from build123d import *

# Parameters (mm, degrees)
SKETCH1_W           = 50
SKETCH1_H           = 12
BOSS_EXTRUDE1_DEPTH = 5
SKETCH2_R           = 2.25
CUT_EXTRUDE1_DEPTH  = 52.662365412
SKETCH3_W           = 2
SKETCH3_H           = 5
CUT_EXTRUDE2_DEPTH  = 52.662365412
CHAMFER1_SIZE       = 1
MOVE_FACE1_BY       = 6.5


with BuildPart() as part:
    # Sketch1 → Boss-Extrude1 (new body)
    with BuildSketch(Plane.XY):
        with Locations((25, 6)):
            Rectangle(SKETCH1_W, SKETCH1_H)
    extrude(amount=BOSS_EXTRUDE1_DEPTH)

    # Sketch2 → Cut-Extrude1 (cut, through all)
    with BuildSketch(Plane.XY.offset(5)):
        with Locations((10, 8.5)):
            Circle(SKETCH2_R)
        with Locations((40, 8.5)):
            Circle(SKETCH2_R)
    extrude(amount=-CUT_EXTRUDE1_DEPTH, mode=Mode.SUBTRACT)

    # Sketch3 → Cut-Extrude2 (cut, through all)
    with BuildSketch(Plane(origin=(50, 0, 0), x_dir=(0, 0, -1), z_dir=(1, 0, 0))):
        with Locations((-4, 2.5)):
            Rectangle(SKETCH3_W, SKETCH3_H)
    extrude(amount=-CUT_EXTRUDE2_DEPTH, mode=Mode.SUBTRACT)

    # Chamfer1
    chamfer1_edges = [part.edges().sort_by_distance(p)[0] for p in [
        (25, 0, 3),
    ]]
    chamfer(chamfer1_edges, length=CHAMFER1_SIZE)

    # Move Face1: a face moved outward by 6.5
    extrude(part.faces().sort_by_distance((25, 8.5, 5))[0], amount=MOVE_FACE1_BY, dir=(0, 0, 1))


solid = part.part
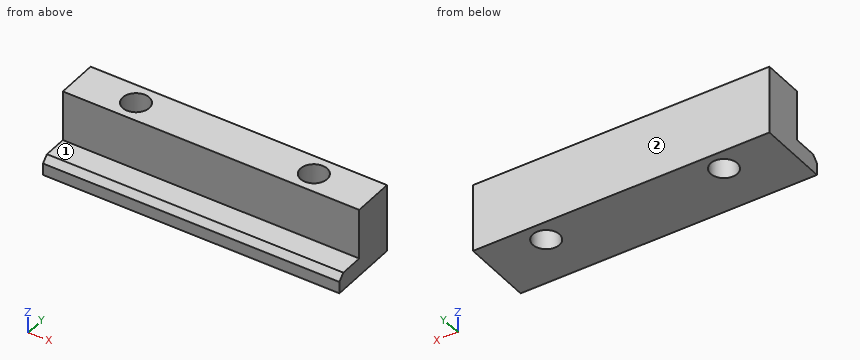
Read the model definition and answer for the solid it produces. Units are mm, in the model's axes. Face numbers are marked on the shaded views. A direction names the side the tool comes from. Round coordinates to 2 decimals unless told otherwise and drop trailing zeros. Write each loop counter-clockwise with the first axis right and the second up, starting at its lowest first coordinate (ties: lowest second). Pieces come first, ordered by that corner, then holes. Notation, with made-up numbers: (2.25, 43.5) - (7.25, 43.5) arc R17 ccw to (7.25, 70.5) - close; hole circle Ø4 at (77.5, 59.25). An arc over 180 degrees is marked (long way). Use a Markdown table: item, result.
(1) The part is cut by section A-A (x = 10). Write down the section's boundary in (y, z), then the cut area to 4 significant figures.
Reported:
| item | result |
|---|---|
| outline | (0, 0) - (6.25, 0) - (6.25, 11.5) - (5, 11.5) - (5, 3) - (1, 3) - (0, 2) - close; (10.75, 0) - (12, 0) - (12, 11.5) - (10.75, 11.5) - close |
| area | 43.25 mm2 |
(2) The part is cut by section C-C (z = 1.25). Write down the section's boundary in (x, y), then the cut area to 3 significant figures.
Reported:
| item | result |
|---|---|
| outline | (0, 0) - (50, 0) - (50, 12) - (0, 12) - close; hole circle Ø4.5 at (10, 8.5); hole circle Ø4.5 at (40, 8.5) |
| area | 568 mm2 |
(3) Which of the six approach directions +Z, -Z, +X, -X, +Y, -Y give full straight-line access (tool end or side, diameter ignored) to the marked faces 1 and 2?
Reported:
| item | result |
|---|---|
| face 1 | +Z, +X, -X, -Y |
| face 2 | +Z, -Z, +X, -X, +Y |
(4) The part is cut by section D-D (x = 30). Write down the section's boundary in (y, z), then the cut area to 3 significant figures.
Reported:
| item | result |
|---|---|
| outline | (0, 0) - (12, 0) - (12, 11.5) - (5, 11.5) - (5, 3) - (1, 3) - (0, 2) - close |
| area | 95.0 mm2 |
(5) Each of these flat-tipped pins is pushed along its axis until it touches: pin 1 Ø5 at (y, z) = (1.5, 8.5) entering from -X; pin 2 Ø5 at (x, y) = (40, 8.5) entering from -Z; pin 3 Ø1.5 at (x, y) = (35, 3.5) entering from +Z. Where does it stop, or does it pass through?
Reported:
| item | result |
|---|---|
| pin 1 | through |
| pin 2 | z = 0 |
| pin 3 | z = 3 |
(6) The part is cut by section B-B (y = 8.5). Write down the section's boundary in (x, z).
Reported:
| item | result |
|---|---|
| outline | (0, 0) - (7.75, 0) - (7.75, 11.5) - (0, 11.5) - close; (12.25, 0) - (37.75, 0) - (37.75, 11.5) - (12.25, 11.5) - close; (42.25, 0) - (50, 0) - (50, 11.5) - (42.25, 11.5) - close |
(7) Straight lines are drawn through the part: line 1 along X through (y, z) = (10.25, 3.25); line 2 along X through (y, z) = (7.75, 2.75); line 3 along Y through (x, z) = (27, 5). For each, find the intervals that lie inside material, in ascending order. Write a range as [from, to].
Reported:
| item | result |
|---|---|
| line 1 | [0, 8.59], [11.41, 38.59], [41.41, 50] |
| line 2 | [0, 7.88], [12.12, 37.88], [42.12, 50] |
| line 3 | [5, 12] |
